from build123d import *

# Parameters (mm, degrees)
EXTRUDE_1_DEPTH      = 88
SKETCH_2_R           = 52.5
EXTRUDE_2_DEPTH      = 18
EXTRUDE_2_TAPER      = 30
SKETCH_3_R           = 2.5
EXTRUDE_3_DEPTH      = 4
SKETCH_4_R           = 52.5
EXTRUDE_4_DEPTH      = 110
SKETCH_5_R           = 45
EXTRUDE_5_DEPTH      = 65
EXTRUDE_6_DEPTH      = 5
EXTRUDE_6_DEPTH_BACK = 5
SKETCH_7_R           = 4
EXTRUDE_7_DEPTH      = 8


with BuildPart() as part:
    # Sketch 1 → Extrude 1 (new body)
    with BuildSketch(Plane.XY):
        with BuildLine():
            Line((100, 0), (100, 90))
            Line((100, 90), (30, 90))
            Line((30, 90), (30, 74.161984871))
            ThreePointArc((30, 74.161984871), (-44.72135955, 66.332495807), (-80, 0))
            ThreePointArc((-80, 0), (10, -90), (100, 0))
        make_face()
    extrude(amount=EXTRUDE_1_DEPTH)

    # Sketch 2 → Extrude 2 (add)
    with BuildSketch(Plane.XY.offset(88)):
        Circle(SKETCH_2_R)
    extrude(amount=EXTRUDE_2_DEPTH, taper=EXTRUDE_2_TAPER)

    # Sketch 3 → Extrude 3 (add)
    with BuildSketch(Plane(origin=(0, 90, 0), x_dir=(1, 0, 0), z_dir=(0, 1, 0))):
        with BuildLine():
            Line((17.5, 13.5), (112.5, 13.5))
            ThreePointArc((112.5, 13.5), (119.571067812, 10.571067812), (122.5, 3.5))
            Line((122.5, 3.5), (122.5, -91.5))
            ThreePointArc((122.5, -91.5), (119.571067812, -98.571067812), (112.5, -101.5))
            Line((112.5, -101.5), (17.5, -101.5))
            ThreePointArc((17.5, -101.5), (10.428932188, -98.571067812), (7.5, -91.5))
            Line((7.5, -91.5), (7.5, 3.5))
            ThreePointArc((7.5, 3.5), (10.428932188, 10.571067812), (17.5, 13.5))
        make_face()
        with Locations(Location((16.5, 4.5, 0), (0, 0, 270))):
            Circle(SKETCH_3_R, mode=Mode.SUBTRACT)
        with Locations(Location((16.5, -92.5, 0), (0, 0, 90))):
            Circle(SKETCH_3_R, mode=Mode.SUBTRACT)
        with Locations(Location((113.5, -92.5, 0), (0, 0, 270))):
            Circle(SKETCH_3_R, mode=Mode.SUBTRACT)
        with Locations(Location((113.5, 4.5, 0), (0, 0, 90))):
            Circle(SKETCH_3_R, mode=Mode.SUBTRACT)
    extrude(amount=EXTRUDE_3_DEPTH)

    # Sketch 4 → Extrude 4 (add)
    with BuildSketch(Plane(origin=(0, 94, 0), x_dir=(1, 0, 0), z_dir=(0, 1, 0))):
        with Locations(Location((65, -44, 0), (0, 0, 90))):
            Circle(SKETCH_4_R)
    extrude(amount=EXTRUDE_4_DEPTH)

    # Sketch 5 → Extrude 5 (add)
    with BuildSketch(Plane(origin=(0, 204, 0), x_dir=(1, 0, 0), z_dir=(0, 1, 0))):
        with Locations(Location((65, -44, 0), (0, 0, 270))):
            Circle(SKETCH_5_R)
    extrude(amount=EXTRUDE_5_DEPTH)



with BuildPart() as body_2:
    # Sketch 6 → Extrude 6 (new, two sides: drawn at the far end of the back side and taken through both)
    with BuildSketch(Plane.ZY.offset(-20).offset(-EXTRUDE_6_DEPTH_BACK)):
        Polygon((44, 239), (39.669872981, 236.5), (39.669872981, 231.5), (44, 229), (48.330127019, 231.5), (48.330127019, 236.5), align=None)
    extrude(amount=EXTRUDE_6_DEPTH + EXTRUDE_6_DEPTH_BACK)


with BuildPart() as part_1:
    add(part.part)

    add(body_2.part)  # Extrude 7 merges body 2
    # Sketch 7 → Extrude 7 (add)
    with BuildSketch(Plane.ZY.offset(-15)):
        with Locations((44, 234)):
            Circle(SKETCH_7_R)
    extrude(amount=EXTRUDE_7_DEPTH)


solid = part_1.part
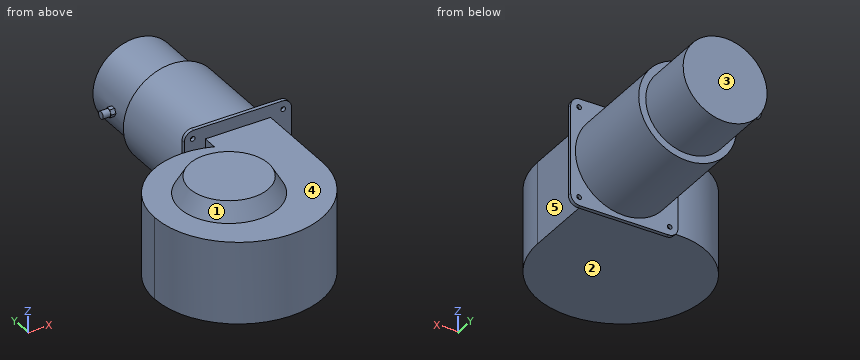
Verification items for the finished model (mm, model axes). Face numbers are marked on the shaded views. A direction names the side the tool comes from. Coordinates: 2 decimals unless noted, no trailing zeros. Loops run counter-clockwise (first coordinate to the right, second up) from the corner with the lowest first, then second, coordinate; pieces in that order, holes last. Notation, with made-up numbers: (58, 17) -> (67, 17) arc R22 ccw to (67, 46) -> close; hole circle Ø3 at (-3.5, 36.5). An arc over 180 degrees is marked (long way). Answer as a JSON object with one key per item and string values. Group by question number.
Item 1: Scan lines: probe 1 along X at (y, z) = (92.05, -4.5); probe 2 along X at (y, z) = (91, -4); probe 3 along Z at (x, y) = (16, 92). Record each from-to range of solid material in increasing order.
Item 2: Mould release check, pull along Y, two halves, no side actions. Record for the marked faces 3, 4 and 5: +Y half, -Y half, draft (parallel to the pull), parting line (faces both ways), or undercut.
Item 3: Tool access check on the marked faces 1 and 2. Record the directions out of +Z, -Z, +X, -X, +Y, -Y that give a thin tool (end or side, any length) a straight path to the whole face; none if there is none.
Item 4: Depth check by flat-ended pin: pin 1 (4 mm diameter, centred on x = 16.5, z = 92.5, fed in from -Y); pin 2 (6 mm diameter, centred on x = -34, y = 44.5, fed in from -Z); pin 3 (5 mm diameter, centred on y = 198, z = 64.5, fed in from +X); pin 4 (3 mm diameter, centred on x = 16.5, z = -4.5, fed in from +Y). Enter the tip coordinate at first touch or a pass-through.
Item 5: Sectioned sample at A-A on z = 55.5. Record the boundary of the cut face in (x, y) (3 decimals).
Item 6: Sectioned sample at D-D on z = 10.5. Record the boundary of the cut face in (x, y), plus the area to 3 significant figures.
Item 7: Sectioned sample at C-C on y = 169. Record the boundary of the cut face in (x, z).
Item 8: Sectioned sample at B-B on x = 80.5. Record the boundary of the cut face in (y, z).
Evaluation:
{
 "1": {"probe 1": "x = 7.55 to 14, 19 to 111, 116 to 122.45", "probe 2": "x = 7.51 to 14.05, 18.95 to 111.05, 115.95 to 122.49", "probe 3": "z = -13.39 to -6.95, -2.05 to 90.05, 94.95 to 101.39"},
 "2": {"face 3": "+Y half", "face 4": "undercut", "face 5": "draft"},
 "3": {"face 1": "+Z", "face 2": "-Z, +X, -X, -Y"},
 "4": {"pin 1": "stops at y = -48.49", "pin 2": "stops at z = 0", "pin 3": "stops at x = 114.32", "pin 4": "passes through"},
 "5": {"outline": "(-80, 0) arc R90 ccw to (100, 0) -> (100, 90) -> (122.5, 90) -> (122.5, 94) -> (116.225, 94) -> (116.225, 204) -> (108.506, 204) -> (108.506, 269) -> (21.494, 269) -> (21.494, 204) -> (13.775, 204) -> (13.775, 94) -> (7.5, 94) -> (7.5, 90) -> (30, 90) -> (30, 74.162) arc R80 ccw to start"},
 "6": {"outline": "(-80, 0) arc R90 ccw to (100, 0) -> (100, 90) -> (122.5, 90) -> (122.5, 94) -> (105.42, 94) -> (105.42, 204) -> (95.05, 204) -> (95.05, 269) -> (34.95, 269) -> (34.95, 204) -> (24.58, 204) -> (24.58, 94) -> (7.5, 94) -> (7.5, 90) -> (30, 90) -> (30, 74.16) arc R80 ccw to start", "area": "39,700 mm²"},
 "7": {"outline": "circle Ø105 at (65, 44)"},
 "8": {"outline": "(-55.94, 0) -> (90, 0) -> (90, -13.5) -> (94, -13.5) -> (94, -6.16) -> (204, -6.16) -> (204, 1.75) -> (269, 1.75) -> (269, 86.25) -> (204, 86.25) -> (204, 94.16) -> (94, 94.16) -> (94, 101.5) -> (90, 101.5) -> (90, 88) -> (-55.94, 88) -> close"}
}
